```python
from build123d import *

# Parameters (mm, degrees)
BASE_PROFILE_SKETCH_W      = 140
BASE_PROFILE_SKETCH_H      = 18
BASE_BLOCK_DEPTH           = 36
UPRIGHT_BLOCK_DEPTH        = 36
GUIDE_RAIL_BOSS_DEPTH      = 30
GUIDE_CAP_BOSS_DEPTH       = 36
SIDE_LUG_DEPTH             = 30
LUG_POCKET_18_DEPTH        = 12
LUG_START                  = -6
LUG_RECESS_18_DEPTH        = 6
LUG_HOLE_SKETCH_R          = 4.5
LUG_HOLE_9_DEPTH           = 12
MOUNTING_PAD_1_25_DEPTH    = 3
MOUNTING_PAD_2_SKETCH_R    = 12.5
MOUNTING_PAD_2_25_DEPTH    = 3
MOUNTING_HOLES_SKETCH_R    = 6
MOUNTING_HOLES_2X_12_DEPTH = 30


with BuildPart() as part:
    # Base Profile Sketch → Base Block (new body)
    with BuildSketch(Plane.XY):
        with Locations((70, 9)):
            Rectangle(BASE_PROFILE_SKETCH_W, BASE_PROFILE_SKETCH_H)
    extrude(amount=BASE_BLOCK_DEPTH)

    # Upright Profile Sketch → Upright Block (add)
    with BuildSketch(Plane.XY.offset(36)):
        Polygon((0, 18), (0, 68), (18, 68), (18, 58), (10, 58), (10, 18), align=None)
    extrude(amount=-UPRIGHT_BLOCK_DEPTH)

    # Guide Rail Sketch → Guide Rail Boss (add)
    with BuildSketch(Plane(origin=(10, 0, 0), x_dir=(0, 0, -1), z_dir=(1, 0, 0))):
        Polygon((-18, 32), (18, 32), (18, 26), (0, 18), (-18, 18), (-36, 18), (-54, 26), (-54, 32), align=None)
    extrude(amount=GUIDE_RAIL_BOSS_DEPTH)

    # Guide Cap Sketch → Guide Cap Boss (add)
    with BuildSketch(Plane(origin=(0, 0, 0), x_dir=(-1, 0, 0), z_dir=(0, 0, -1))):
        Polygon((-40, 18), (-50, 18), (-50, 68), (-32, 68), (-32, 58), (-40, 58), align=None)
    extrude(amount=-GUIDE_CAP_BOSS_DEPTH)

    # Side Lug Sketch → Side Lug (add)
    with BuildSketch(Plane(origin=(0, 0, 0), x_dir=(-1, 0, 0), z_dir=(0, 0, -1))):
        with BuildLine():
            Line((0, 0), (0, 18))
            Line((0, 18), (10, 18))
            Line((10, 18), (11, 18))
            ThreePointArc((11, 18), (20, 9), (11, 0))
            Line((11, 0), (0, 0))
        make_face()
    extrude(amount=-SIDE_LUG_DEPTH)

    # Lug Pocket Sketch → Lug Pocket Ø18 (cut)
    with BuildSketch(Plane(origin=(0, 0, 0), x_dir=(-1, 0, 0), z_dir=(0, 0, -1))):
        with BuildLine():
            Line((0, 18), (11, 18))
            ThreePointArc((11, 18), (20, 9), (11, 0))
            Line((11, 0), (0, 0))
            Line((0, 0), (0, 18))
        make_face()
    extrude(amount=-LUG_POCKET_18_DEPTH, mode=Mode.SUBTRACT)

    # Lug Recess Sketch → Lug Recess Ø18 (cut)
    with BuildSketch(Plane.XY.offset(30).offset(LUG_START)):
        with BuildLine():
            Line((0, 18), (-11, 18))
            ThreePointArc((-11, 18), (-20, 9), (-11, 0))
            Line((-11, 0), (0, 0))
            Line((0, 0), (0, 18))
        make_face()
    extrude(amount=LUG_RECESS_18_DEPTH, mode=Mode.SUBTRACT)

    # Lug Hole Sketch → Lug Hole Ø9 (cut)
    with BuildSketch(Plane.XY.offset(24)):
        with Locations((-11, 9)):
            Circle(LUG_HOLE_SKETCH_R)
    extrude(amount=-LUG_HOLE_9_DEPTH, mode=Mode.SUBTRACT)

    # Mounting Pad 1 Sketch → Mounting Pad 1 Ø25 (add)
    with BuildSketch(Plane(origin=(0, 18, 0), x_dir=(1, 0, 0), z_dir=(0, 1, 0))):
        with BuildLine():
            Line((60, -5.5), (50, -5.5))
            Line((50, -5.5), (50, -30.5))
            Line((50, -30.5), (60, -30.5))
            ThreePointArc((60, -30.5), (72.5, -18), (60, -5.5))
        make_face()
    extrude(amount=MOUNTING_PAD_1_25_DEPTH)

    # Mounting Pad 2 Sketch → Mounting Pad 2 Ø25 (add)
    with BuildSketch(Plane(origin=(0, 18, 0), x_dir=(1, 0, 0), z_dir=(0, 1, 0))):
        with Locations(Location((120, -18, 0), (0, 0, 90))):
            Circle(MOUNTING_PAD_2_SKETCH_R)
    extrude(amount=MOUNTING_PAD_2_25_DEPTH)

    # Mounting Holes Sketch → Mounting Holes 2xØ12 (cut)
    with BuildSketch(Plane(origin=(0, 21, 0), x_dir=(1, 0, 0), z_dir=(0, 1, 0))):
        with Locations(Location((120, -18, 0), (0, 0, 270))):
            Circle(MOUNTING_HOLES_SKETCH_R)
        with Locations(Location((60, -18, 0), (0, 0, 270))):
            Circle(MOUNTING_HOLES_SKETCH_R)
    extrude(amount=-MOUNTING_HOLES_2X_12_DEPTH, mode=Mode.SUBTRACT)


solid = part.part
```
The model under review builds one solid part; all positions refer to its coordinate system, in mm. A direction names the side the tool comes from. Round coordinates to 2 decimals unless told otherwise and drop trailing zeros. Write each loop counter-clockwise with the first axis right and the second up, starting at its lowest first coordinate (ties: lowest second). Pieces come first, ordered by that corner, then holes.
(1) We need section C-C on x = 110. Give the boundary of the cut face in (y, z), and give its area (3 significant figures).
(2) We need section A-A on y = 9. Give the boundary of the cut face in (x, z), and give its area (3 significant figures).
(3) Machinability: for faces 4 (the flat face through (-6, 9, 24)), 5 (the cylindrical face through (-6.708, 10.352, 18.084)), 6 (the flat face through (40, 27, -7)), 7 (the flat face through (55, 19, 5.5)), 8 (the flat face through (125.4, 21, 21)), which of the approach directions +Z, -Z, +X, -X, +Y, -Y give a long, thin tool a straight path to every point of the face, cutting with its end or side? Answer none if there is none.
(4) We need section B-B on z = 18. Give the number of separate pieces and of enclosed holes in the cut face, and give its area (3 significant figures).
(5) Insertion check: pin 1 (8 mm diameter, centred on x = 40.5, y = 17, fed in from -Z); pin 2 (9 mm diameter, centred on x = -5, y = 7.5, fed in from -Z); pin 3 (4 mm diameter, centred on y = 47.5, z = 21.5, fed in from -X); pin 4 (5 mm diameter, centred on x = 31, z = 31, fed in from -Y). Each pin has a flat end and moves straight along its axis. Give the tip position at first contact, or say it passes through.
(6) We need section D-D on y = 28. Give the boundary of the cut face in (x, z), and give its area (3 significant figures).
(7) Wall thickness on L1, parallel to X at y = 37, z = 26; L2, parallel to Y at x = -11, z = 16; L3, parallel to X at y = 7.25, z = 18: over which ranges is each line inside the solid? List them lowest first.
(8) Mouldability with a two-part tool opening along Z and no side actions: class faces 1 (the flat face through (18, 63, 18)), 2 (the cylindrical face through (57.7, 10.65, 23.54)), 3 (the flat face through (54, 17, 36)) as +Z half, -Z half, draft (parallel to the pull), parting line (faces both ways), or undercut.
Findings below:
1. outline: (0, 0) - (18, 0) - (18, 10.5) - (21, 10.5) - (21, 25.5) - (18, 25.5) - (18, 36) - (0, 36) - close
1. area: 693 mm2
2. outline: (-20, 12) - (-15.5, 12) - (-15.5, 24) - (-20, 24) - close; (-6.5, 12) - (0, 12) - (0, 0) - (140, 0) - (140, 36) - (0, 36) - (0, 24) - (-6.5, 24) - close; hole circle Ø12 at (60, 18); hole circle Ø12 at (120, 18)
2. area: 4,950 mm2
3. face 4: +Z, -X, +Y, -Y
3. face 5: +Z, -Z
3. face 6: -Z, +X, +Y, -Y
3. face 7: -Z, +X, +Y
3. face 8: +Z, -Z, +X, +Y
4. separate pieces: 3
4. enclosed holes: 1
4. area: 4,000 mm2
5. pin 1: stops at z = -6.68
5. pin 2: stops at z = 12
5. pin 3: stops at x = 0
5. pin 4: stops at y = 0
6. outline: (0, 0) - (10, 0) - (10, -18) - (40, -18) - (40, 0) - (50, 0) - (50, 36) - (40, 36) - (40, 54) - (10, 54) - (10, 36) - (0, 36) - close
6. area: 2,880 mm2
7. L1: x = 0 to 10, 40 to 50
7. L2: y = 0 to 4.5, 13.5 to 18
7. L3: x = -19.83 to -15.15, -6.85 to 54, 66 to 114, 126 to 140
8. face 1: draft
8. face 2: undercut
8. face 3: +Z half
